Geometry check sheet. Reference: drawing and pictorial views, mm from the part's lowest x, y, z. A direction names the side the tool comes from. Coordinates: 2 decimals unless noted, no trailing zeros. Loops run counter-clockwise (first coordinate to the right, second up) from the corner with the lowest first, then second, coordinate; pieces in that order, holes last.
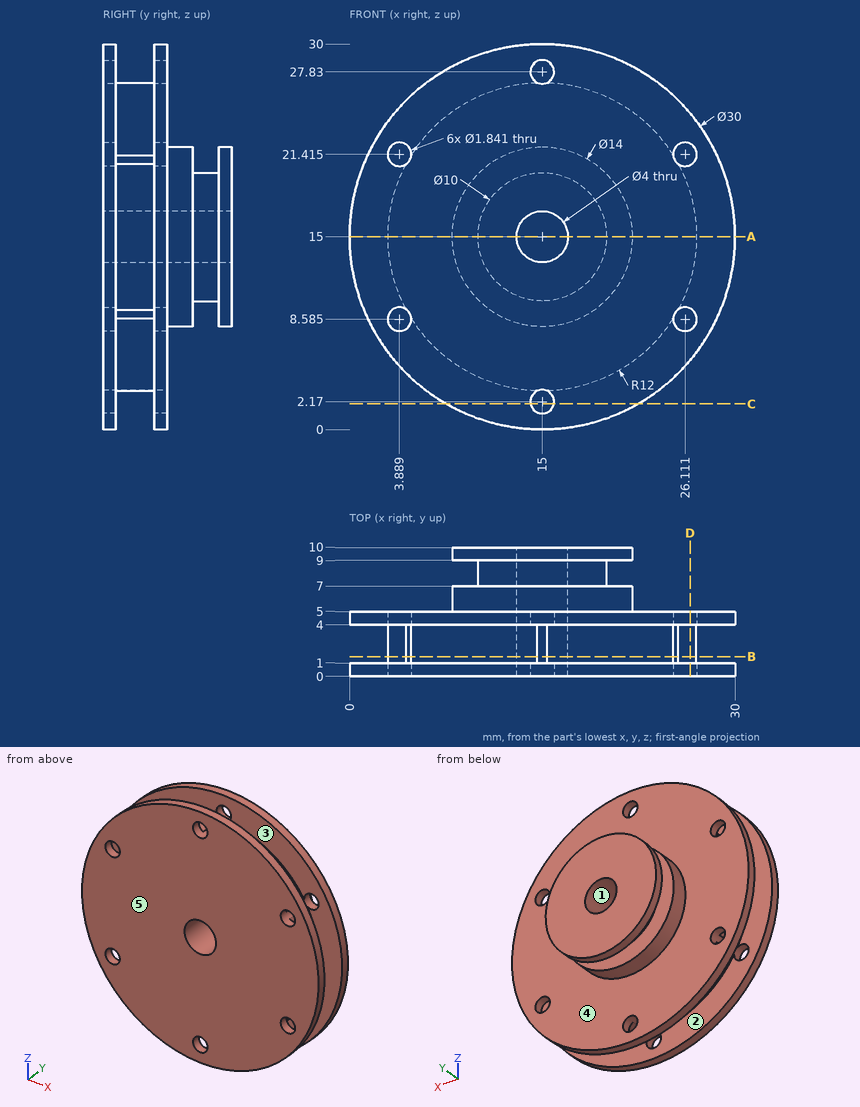
1) Material ranges on probe 1 along Y at (x, z) = (21.5, 27); probe 2 along Y at (x, z) = (7, 7); probe 3 along Z at (x, y) = (3.75, 4.25) (1 decimal), recorded low to high.
Data:
probe 1: y = 0 to 1, 4 to 5
probe 2: y = 0 to 5
probe 3: z = 5.1 to 7.7, 9.5 to 20.5, 22.3 to 24.9
2) Section check A-A on z = 15. Record the cut outline in (x, y), and give its area (3 significant figures).
Data:
outline: (0, 0) - (13, 0) - (13, 10) - (8, 10) - (8, 9) - (10, 9) - (10, 7) - (8, 7) - (8, 5) - (0, 5) - (0, 4) - (3, 4) - (3, 1) - (0, 1) - close; (17, 0) - (30, 0) - (30, 1) - (27, 1) - (27, 4) - (30, 4) - (30, 5) - (22, 5) - (22, 7) - (20, 7) - (20, 9) - (22, 9) - (22, 10) - (17, 10) - close
area: 154 mm2
3) Section check C-C on z = 2. Record the cut outline in (x, y) (1 decimal), and give its area (3 significant figures).
Data:
outline: (7.5, 0) - (14.1, 0) - (14.1, 1) - (7.5, 1) - close; (7.5, 4) - (14.1, 4) - (14.1, 5) - (7.5, 5) - close; (15.9, 0) - (22.5, 0) - (22.5, 1) - (15.9, 1) - close; (15.9, 4) - (22.5, 4) - (22.5, 5) - (15.9, 5) - close
area: 26.3 mm2
4) Depth check by flat-ended pin: pin 1 (2.5 mm diameter, centred on x = 26.11, z = 8.59, fed in from +Y); pin 2 (3 mm diameter, centred on y = 5.5, z = 5.5, fed in from +X); pin 3 (2 mm diameter, centred on y = 8.5, z = 12, fed in from -X). Enter the tip coordinate at first touch or a pass-through.
Data:
pin 1: stops at y = 5
pin 2: stops at x = 27.63
pin 3: stops at x = 8.33
5) Section check B-B on y = 1.5. Record the cut outline in (x, z) (1 decimal), and give its area (3 significant figures).
Data:
outline: (4.4, 9.3) arc R0.9 cw to (4.8, 8.7) arc R12 ccw to (14.6, 3) arc R0.9 cw to (15.4, 3) arc R12 ccw to (25.2, 8.7) arc R0.9 cw to (25.6, 9.3) arc R12 ccw to (25.6, 20.7) arc R0.9 cw to (25.2, 21.3) arc R12 ccw to (15.4, 27) arc R0.9 cw to (14.6, 27) arc R12 ccw to (4.8, 21.3) arc R0.9 cw to (4.4, 20.7) arc R12 ccw to start; hole circle Ø4 at (15, 15)
area: 440 mm2
6) Section check D-D on x = 26.5. Record the cut outline in (y, z), and give its area (3 significant figures).
Data:
outline: (0, 5.37) - (1, 5.37) - (1, 7.75) - (0, 7.75) - close; (0, 9.42) - (1, 9.42) - (1, 11.57) - (4, 11.57) - (4, 9.42) - (5, 9.42) - (5, 20.58) - (4, 20.58) - (4, 18.43) - (1, 18.43) - (1, 20.58) - (0, 20.58) - close; (0, 22.25) - (1, 22.25) - (1, 24.63) - (0, 24.63) - close; (4, 5.37) - (5, 5.37) - (5, 7.75) - (4, 7.75) - close; (4, 22.25) - (5, 22.25) - (5, 24.63) - (4, 24.63) - close
area: 52.4 mm2
7) Access from +Z, -Z, +X, -X, +Y, -Y to the whole of each face (thin tool, end or side, straight path). Record for the marked faces 3, 4 and 5.
Data:
face 3: none
face 4: +Y
face 5: +Z, -Z, +X, -X, -Y
8) Mould release check, pull along Z, two halves, no side actions. Record for the marked faces 1 and 2: +Z half, -Z half, draft (parallel to the pull), parting line (faces both ways), or undercut.
Data:
face 1: undercut
face 2: draft
